Read the model definition and answer for the solid it produces. Units are mm, in the model's axes. A direction names the side the tool comes from. Coordinates: 2 decimals unless noted, no trailing zeros. Write each loop counter-clockwise with the first axis right and the second up, starting at its lowest first coordinate (ties: lowest second). Pieces come first, ordered by that corner, then holes. Notation, with made-up numbers: M 23.5,-6.75 L 33.5,-6.75 A22 ccw 33.5,31.25 Z; hole C 41.5,17 d4. An arc over 180 degrees is marked long. Use a Markdown table: item, result. Add a question column.
from build123d import *

# Parameters (mm, degrees)
SKETCH_1_W             = 35
SKETCH_1_H             = 50
EXTRUDE_1_DEPTH        = 7.5
CUT_EXTRUDE_1_DEPTH    = 35.003676272
HOLE_WIZARD_M4_2_D     = 3.3
CHAMFER_1_SIZE         = 1
HOLE_WIZARD_M6_1_D     = 5
HOLE_WIZARD_M6_1_DEPTH = 15
HOLE_WIZARD_M6_1_TIP   = 1.502151548
SKETCH_17_W            = 12
SKETCH_17_H            = 6
CUT_EXTRUDE_2_DEPTH    = 35.003676272
SKETCH_19_W            = 21
SKETCH_19_H            = 6
CUT_EXTRUDE_8_DEPTH    = 35.003676272


with BuildPart() as part:
    # 草图1 → 凸台-拉伸1 (new, symmetric)
    with BuildSketch(Plane.XY):
        Rectangle(SKETCH_1_W, SKETCH_1_H)
    extrude(amount=EXTRUDE_1_DEPTH, both=True)

    # 草图2 → 切除-拉伸1 (cut, through all)
    with BuildSketch(Plane.XY.offset(7.5)):
        with BuildLine():
            Line((-17.5, 6.75), (-12.5, 6.75))
            ThreePointArc((-12.5, 6.75), (-5.75, 0), (-12.5, -6.75))
            Line((-12.5, -6.75), (-17.5, -6.75))
            ThreePointArc((-17.5, -6.75), (-24.25, 0), (-17.5, 6.75))
        make_face()
    extrude(amount=-CUT_EXTRUDE_1_DEPTH, mode=Mode.SUBTRACT)

    # M4 螺纹孔2 (through all)
    with Locations(Plane(origin=(0, 0, -7.5), x_dir=(-1, 0, 0), z_dir=(0, 0, -1))):
        with Locations((4, -14), (13, -14), (4, 14), (13, 14)):
            Hole(HOLE_WIZARD_M4_2_D / 2)

    # 倒角1
    chamfer_1_edges = [part.edges().sort_by_distance(p)[0] for p in [
        (-17.5, -6.75, 0),
        (-17.5, 6.75, 0),
        (17.5, -25, 0),
        (17.5, 25, 0),
    ]]
    chamfer(chamfer_1_edges, length=CHAMFER_1_SIZE)

    # M6 螺纹孔1
    with Locations(Plane(origin=(17.5, 0, 0), x_dir=(0, 0, -1), z_dir=(1, 0, 0))):
        with Locations((0, -17.5), (0, 17.5)):
            Hole(HOLE_WIZARD_M6_1_D / 2, depth=HOLE_WIZARD_M6_1_DEPTH)
            with Locations((0, 0, -(HOLE_WIZARD_M6_1_DEPTH + HOLE_WIZARD_M6_1_TIP / 2))):  # 118° drill point
                Cone(0, HOLE_WIZARD_M6_1_D / 2, HOLE_WIZARD_M6_1_TIP, mode=Mode.SUBTRACT)

    # 草图17 → 切除-拉伸2 (cut, through all)
    with BuildSketch(Plane.XY.offset(7.5)):
        with Locations((11.5, 0)):
            Rectangle(SKETCH_17_W, SKETCH_17_H)
    extrude(amount=-CUT_EXTRUDE_2_DEPTH, mode=Mode.SUBTRACT)

    # 草图19 → 切除-拉伸8 (cut, through all)
    with BuildSketch(Plane.XY.offset(7.5)):
        with Locations((-7, -22)):
            Rectangle(SKETCH_19_W, SKETCH_19_H)
        with Locations((-7, 22)):
            Rectangle(SKETCH_19_W, SKETCH_19_H)
    extrude(amount=-CUT_EXTRUDE_8_DEPTH, mode=Mode.SUBTRACT)


solid = part.part
Item 1: Determine the mould class of faces 1 (the cylindrical face through (-5.216, -12.885, 0.105)), 2 (the conical face through (1.259, 17.076, 0.094)), 3 (the flat face through (4, 0, 7.5)) for opening direction Z: pulls with the +Z half, pulls with the -Z half, needs draft (parallel to the pull), parting line crosses it, or undercut.
Item 2: Find section B-B on x = -4. Give the vertices of the cut face in (y, z), then the cut area to 3 significant figures.
Item 3: For faces 4 (the flat face through (5.5, 0, 0)), 5 (the flat face through (-16.99, -7.24, 0.1)), 6 (the cylindrical face through (9.9, -15.39, 1.34)), determine the directions among +Z, -Z, +X, -X, +Y, -Y from which every point of the face is accessible in a straight line to the end or side of a thin tool.
Item 4: Find section C-C on y = 14. Give the vertices of the cut face in (x, z).
Item 5: Each of these flat-tipped pins is pushed along its axis until it touches: pin 1 (5 mm diameter, centred on y = 22.5, z = 2.5, fed in from -X); pin 2 (3 mm diameter, centred on y = 0.5, z = -2, fed in from +X); pin 3 (4 mm diameter, centred on x = -4, y = 14, fed in from -Z); pin 4 (6 mm diameter, centred on x = -6.5, z = -1, fed in from -Y). Where does it stop, or does it pass through?
Item 6: Find section D-D on z = -3.5. Give the vertices of the cut face in (x, y).
Item 7: Find section A-A on x = 9. Give the vertices of the cut face in (y, z), then the cut area to 3 significant figures.
Item 8: Consider probe 1 along Y at (x, z) = (-13, -2); probe 2 along Y at (x, z) = (-15, 2.5); probe 3 along Y at (x, z) = (13.5, -4). Determine where each line is inside the solid, lowest interval first.
Geometry says:
| question | item | result |
|---|---|---|
| 1 | face 1 | needs draft |
| 1 | face 2 | undercut |
| 1 | face 3 | pulls with the +Z half |
| 2 | outline | M -19,-7.5 L -15.65,-7.5 L -15.65,7.5 L -19,7.5 Z; M -12.35,-7.5 L 12.35,-7.5 L 12.35,7.5 L -12.35,7.5 Z; M 15.65,-7.5 L 19,-7.5 L 19,7.5 L 15.65,7.5 Z |
| 2 | area | 471 mm2 |
| 3 | face 4 | +Z, -Z, +X |
| 3 | face 5 | +Z, -Z, -X |
| 3 | face 6 | +X |
| 4 | outline | M -17.5,-7.5 L -14.65,-7.5 L -14.65,7.5 L -17.5,7.5 Z; M -11.35,-7.5 L -5.65,-7.5 L -5.65,7.5 L -11.35,7.5 Z; M -2.35,-7.5 L 17.5,-7.5 L 17.5,7.5 L -2.35,7.5 Z |
| 5 | pin 1 | stops at x = 3.5 |
| 5 | pin 2 | stops at x = 5.5 |
| 5 | pin 3 | stops at z = -7.5 |
| 5 | pin 4 | stops at y = -19 |
| 6 | outline | M -17.5,-19 L 3.5,-19 L 3.5,-25 L 16.5,-25 L 17.5,-24 L 17.5,-3 L 5.5,-3 L 5.5,3 L 17.5,3 L 17.5,24 L 16.5,25 L 3.5,25 L 3.5,19 L -17.5,19 L -17.5,7.75 L -16.5,6.75 L -12.5,6.75 A6.75 cw -12.5,-6.75 L -16.5,-6.75 L -17.5,-7.75 Z; hole C -13,-14 d3.3; hole C -13,14 d3.3; hole C -4,-14 d3.3; hole C -4,14 d3.3 |
| 7 | outline | M -25,-7.5 L -3,-7.5 L -3,7.5 L -25,7.5 Z; M 3,-7.5 L 25,-7.5 L 25,7.5 L 3,7.5 Z; hole C -17.5,0 d5; hole C 17.5,0 d5 |
| 7 | area | 621 mm2 |
| 8 | probe 1 | y = -19 to -15.65, -12.35 to -6.75, 6.75 to 12.35, 15.65 to 19 |
| 8 | probe 2 | y = -19 to -6.75, 6.75 to 19 |
| 8 | probe 3 | y = -25 to -3, 3 to 25 |
